Read the model definition and answer for the solid it produces. Units are mm, in the model's axes. Face numbers are marked on the shaded views. Round coordinates to 2 decimals unless told otherwise and drop trailing zeros. Write each loop counter-clockwise with the first axis right and the second up, starting at its lowest first coordinate (ties: lowest second). Pieces come first, ordered by that corner, then holes.
from build123d import *

# Parameters (mm, degrees)
HEX_PROFILE_WITH_BORE_12_R = 6
HEX_BODY_15MM_DEPTH        = 15


with BuildPart() as part:
    # Hex Profile with Bore Ø12 → Hex Body 15mm (new body)
    with BuildSketch(Plane.XY):
        Polygon((12, 0), (6, 10.392304845), (-6, 10.392304845), (-12, 0), (-6, -10.392304845), (6, -10.392304845), align=None)
        Circle(HEX_PROFILE_WITH_BORE_12_R, mode=Mode.SUBTRACT)
    extrude(amount=HEX_BODY_15MM_DEPTH)


solid = part.part
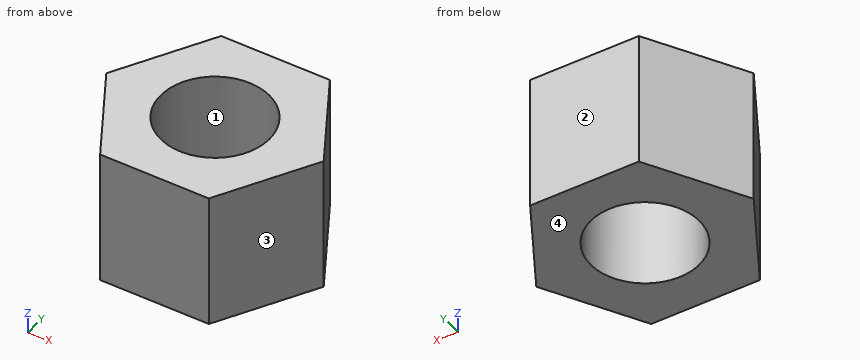
Q1. Flat-ended cylindrical pins translate along their axes: pin 1 Ø2 at (y, z) = (7, 7) entering from -X; pin 2 Ø4 at (x, z) = (9.5, 11.5) entering from +Y; pin 3 Ø6 at (x, y) = (-0.5, -2) entering from -Z; pin 4 Ø8 at (y, z) = (-6.5, 12.5) entering from -X. Find the tip coordinate at first contact, or state that the pin passes through.
Verdict:
pin 1: stops at x = -8.54
pin 2: stops at y = 7.79
pin 3: passes through
pin 4: stops at x = -10.56
Q2. Section A-A (x = 0) is taken. Determine the outline of the cut face in (y, z), then the cut area to 3 significant figures.
Verdict:
outline: (-10.39, 0) - (-6, 0) - (-6, 15) - (-10.39, 15) - close; (6, 0) - (10.39, 0) - (10.39, 15) - (6, 15) - close
area: 132 mm2
Q3. Section B-B (y = -2) is taken. Determine the outline of the cut face in (x, z).
Verdict:
outline: (-10.85, 0) - (-5.66, 0) - (-5.66, 15) - (-10.85, 15) - close; (5.66, 0) - (10.85, 0) - (10.85, 15) - (5.66, 15) - close
Q4. Section C-C (z = 11) is taken. Determine the outline of the cut face in (x, y), then the cut area to 3 significant figures.
Verdict:
outline: (-12, 0) - (-6, -10.39) - (6, -10.39) - (12, 0) - (6, 10.39) - (-6, 10.39) - close; hole circle Ø12 at (0, 0)
area: 261 mm2
Q5. Straight lines are drawn through the part: probe 1 along Y at (x, z) = (0, 9.5); probe 2 along X at (y, z) = (0.75, 10.25); probe 3 along X at (y, z) = (-1.25, 11.25). For each, find the intervals that lie inside material, in ascending order.
Verdict:
probe 1: y = -10.39 to -6, 6 to 10.39
probe 2: x = -11.57 to -5.95, 5.95 to 11.57
probe 3: x = -11.28 to -5.87, 5.87 to 11.28
Q6. Determine the mould class of the marked faces 1, 2, 3 and 4 for opening direction Y: pulls with the +Y half, pulls with the -Y half, needs draft (parallel to the pull), parting line crosses it, or undercut.
Verdict:
face 1: undercut
face 2: pulls with the +Y half
face 3: pulls with the -Y half
face 4: needs draft
Q7. Section D-D (y = 8) is taken. Determine the outline of the cut face in (x, z), then the cut area to 3 significant figures.
Verdict:
outline: (-7.38, 0) - (7.38, 0) - (7.38, 15) - (-7.38, 15) - close
area: 221 mm2
